```python
from build123d import *

# Parameters (mm, degrees)
EXTRUDE_1_DEPTH = 300


with BuildPart() as part:
    # 草图1 → 凸台-拉伸1 (new, symmetric)
    with BuildSketch(Plane.XY):
        Polygon((0, 0), (0, 100), (250, 100), (250, 300), (600, 300), (600, 0), align=None)
    extrude(amount=EXTRUDE_1_DEPTH, both=True)


solid = part.part
```
Input: part model. Units: mm. Frame: model coordinates. A direction names the side the tool comes from. Round coordinates to 2 decimals unless told otherwise and drop trailing zeros. Loops run counter-clockwise (first coordinate to the right, second up) from the corner with the lowest first, then second, coordinate; pieces in that order, holes last. Notation, with made-up numbers: (79.25, 80.5) -> (102.25, 80.5) arc R30 cw to (102.25, 107.5) -> close; hole circle Ø6 at (-7, 3). An arc over 180 degrees is marked (long way). Use one line per item in the form item = value. Start each with the question number.
Item 1: Material intervals for L1, parallel to X at y = 114, z = 167; L2, parallel to Y at x = 209, z = -212.5, sorted ascending. Write a range as from..to.
Item 2: Section query B-B on x = 51. Return the cut outline in (y, z).
Item 3: Set-up query: faces 1 (the face through (123, 100, 4)), 2 (the face through (371, 119, 300)). Return all of +Z, -Z, +X, -X, +Y, -Y with unobstructed straight access to the full face (end or side cutting, diameter ignored); none if empty.
Item 4: Contact query for flat-ended pins moving along their axis: pin 1 Ø5 at (x, z) = (150.5, 209) entering from -Y; pin 2 Ø4 at (x, z) = (199, -100.5) entering from +Y. Output: stop coordinate, or through.
Item 5: Section query A-A on z = -20.5. Return the cut outline in (x, y), then the cut area to 3 significant figures.
Item 6: Mould query, pull axis X, two halves, no side actions, for faces 3 (the face through (0, 49, 4)), 4 (the face through (423, 300, 4)), 5 (the face through (600, 152, 4)). Classes: pulls with the +X half, pulls with the -X half, needs draft (parallel to the pull), parting line crosses it, or undercut.
Item 7: Section query C-C on y = 261. Return the cut outline in (x, z).
Ans:
q1.L1 = 250..600
q1.L2 = 0..100
q2.outline = (0, -300) -> (100, -300) -> (100, 300) -> (0, 300) -> close
q3.face_1 = +Z, -Z, -X, +Y
q3.face_2 = +Z, +X, -X, +Y, -Y
q4.pin_1 = 0
q4.pin_2 = 100
q5.outline = (0, 0) -> (600, 0) -> (600, 300) -> (250, 300) -> (250, 100) -> (0, 100) -> close
q5.area = 130,000 mm^2
q6.face_3 = pulls with the -X half
q6.face_4 = needs draft
q6.face_5 = pulls with the +X half
q7.outline = (250, -300) -> (600, -300) -> (600, 300) -> (250, 300) -> close
